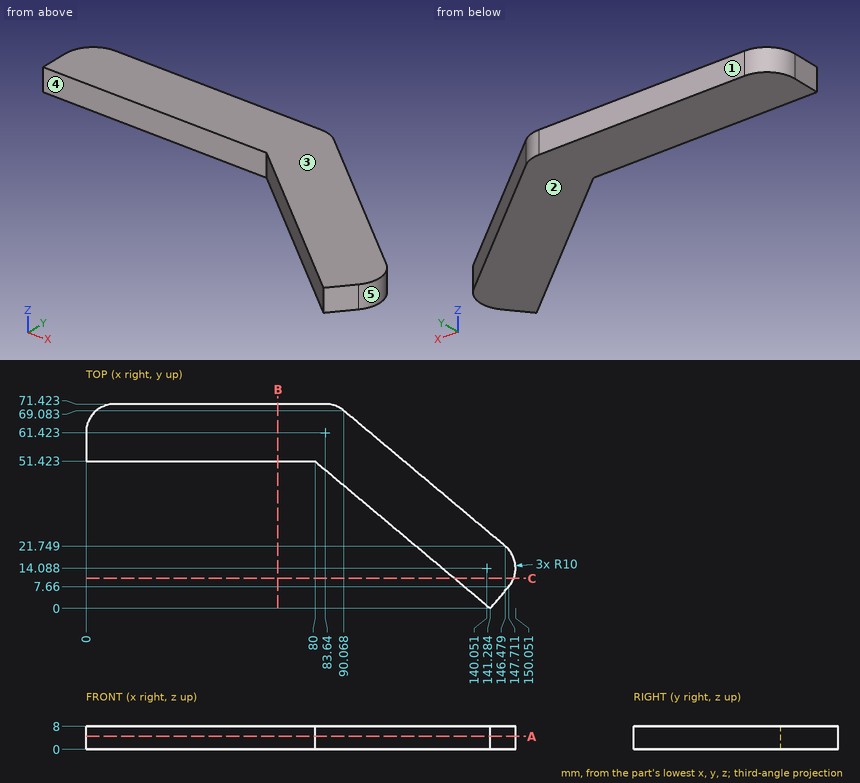
Study the drawing (mm; zero at the part's minimum x, y, z) and answer. A direction names the side the tool comes from. Give positions to 0.01 mm unless a question says otherwise; leave off trailing zeros. Order: outer loops, then holes, each group sorted by start corner. A loop starts at its lowest first (then second) coordinate and runs counter-clockwise, first axis right, second up. Notation, with made-up numbers: M 57,-0.75 L 73,-0.75 A32 cw 73,31.25 Z; hole C 8.25,-1 d11. An arc over 180 degrees is marked long. Put each result on its own line as item: value. Start each with the question number.
Item 1: Which of the six approach directions +Z, -Z, +X, -X, +Y, -Y give full straight-line access (tool end or side, diameter ignored) to the marked faces 4 and 5?
Item 2: The part is cut by section C-C, the plane y = 10.5. Determine the outline of the cut face in (x, z) (1 decimal).
Item 3: The part is cut by section A-A, the plane z = 4.5. Determine the outline of the cut face in (x, y).
Item 4: For a pull along Z with two mould halves and no side action, classify the marked faces 1, 2 and 3 as +Z half, -Z half, draft (parallel to the pull), parting line (faces both ways), or undercut.
Item 5: Flat-ended cylindrical pins translate along their axes: P1, Ø4, axis at x = 53.5, z = 4, coming from the -Y side; P2, Ø4, axis at x = 95.5, z = 5.5, coming from the +Y side; P3, Ø12, axis at x = 49, y = 48.5, coming from the +Z side; P4, Ø1.5, axis at x = 123.5, z = 6.5, coming from the -Y side. Find the tip coordinate at first contact, or state that the pin passes through.
Item 6: The part is cut by section B-B, the plane x = 67. Determine the outline of the cut face in (y, z).
Item 7: Find the intervals of material crossed by line 1 along Y through (x, z) = (77.5, 6.25); line 2 along X through (y, z) = (38, 2.75) (1 decimal); line 3 along X through (y, z) = (47, 6.25) (1 decimal), in increasing order.
Answer key:
1. face 4: +Z, -Z, -X, -Y
1. face 5: +Z, -Z, +X
2. outline: M 128.8,0 L 149.4,0 L 149.4,8 L 128.8,8 Z
3. outline: M 0,51.42 L 80,51.42 L 141.28,0 L 147.71,7.66 A10 ccw 146.48,21.75 L 90.07,69.08 A10 ccw 83.64,71.42 L 10,71.42 A10 ccw 0,61.42 Z
4. face 1: draft
4. face 2: -Z half
4. face 3: +Z half
5. P1: stops at y = 51.42
5. P2: stops at y = 66.2
5. P3: stops at z = 8
5. P4: stops at y = 14.29
6. outline: M 51.42,0 L 71.42,0 L 71.42,8 L 51.42,8 Z
7. line 1: y = 51.42 to 71.42
7. line 2: x = 96 to 127.1
7. line 3: x = 85.3 to 116.4
